from build123d import *

# Parameters (mm, degrees)
EXTRUDE_1_DEPTH     = 45
CUT_EXTRUDE_1_DEPTH = 63.24949799
FILLET_1_R          = 2
FILLET_2_R          = 7
CHAMFER_1_SIZE      = 1


with BuildPart() as part:
    # 草图1 → 拉伸-薄壁1 (new body)
    with BuildSketch(Plane.XY):
        Polygon((0, 0), (0, 30), (35, 30), (35, 25), (5, 25), (5, 0), align=None)
    extrude(amount=EXTRUDE_1_DEPTH)

    # 草图2 → 切除-拉伸1 (cut, through all)
    with BuildSketch(Plane.XZ.offset(-25)):
        with BuildLine():
            Line((27, 35), (27, 10))
            ThreePointArc((27, 10), (22.5, 5.5), (18, 10))
            Line((18, 10), (18, 35))
            ThreePointArc((18, 35), (22.5, 39.5), (27, 35))
        make_face()
    extrude(amount=-CUT_EXTRUDE_1_DEPTH, mode=Mode.SUBTRACT)

    # 圆角1
    fillet_1_edges = [part.edges().sort_by_distance(p)[0] for p in [
        (5, 25, 22.5),
    ]]
    fillet(fillet_1_edges, radius=FILLET_1_R)

    # 圆角2
    fillet_2_edges = [part.edges().sort_by_distance(p)[0] for p in [
        (0, 30, 22.5),
    ]]
    fillet(fillet_2_edges, radius=FILLET_2_R)

    # 倒角1
    chamfer_1_edges = [part.edges().sort_by_distance(p)[0] for p in [
        (2.5, 0, 45),
        (2.5, 0, 0),
        (35, 27.5, 0),
        (35, 27.5, 45),
    ]]
    chamfer(chamfer_1_edges, length=CHAMFER_1_SIZE)


solid = part.part
Design review of the part built by this model. Coordinates are the model's own, in mm. A direction names the side the tool comes from. Give positions to 0.01 mm unless a question says otherwise; leave off trailing zeros. Loops run counter-clockwise (first coordinate to the right, second up) from the corner with the lowest first, then second, coordinate; pieces in that order, holes last. Notation, with made-up numbers: M 50.25,33.5 L 56.25,33.5 A33 ccw 56.25,63.5 Z; hole C -35,12 d7. An arc over 180 degrees is marked long. Answer as a JSON object with one key per item and string values.
Item 1: We need section A-A (x = 22.5). State the section outline as (y, z) points, and give its area (3 significant figures).
Output values:
{"outline": "M 25,0 L 30,0 L 30,5.5 L 25,5.5 Z; M 25,39.5 L 30,39.5 L 30,45 L 25,45 Z", "area": "55.0 mm2"}
Item 2: Machinability: for faces 5 (the face through (18, 27, 22)), 6 (the face through (3, 0, 22)), 7 (the face through (15, 25, 22)), which of the approach directions +Z, -Z, +X, -X, +Y, -Y give a long, thin tool a straight path to every point of the face, cutting with its end or side? Answer none if there is none.
Output values:
{"face 5": "+Y, -Y", "face 6": "+Z, -Z, +X, -X, -Y", "face 7": "+Z, -Z, +X, -Y"}
Item 3: We need section C-C (y = 4.5). State the section outline as (x, z) points.
Output values:
{"outline": "M 0,0 L 5,0 L 5,45 L 0,45 Z"}
Item 4: Mouldability with a two-part tool opening along Z and no side actions: class faces 1 (the face through (12, 26, 0)), 2 (the face through (22.4, 27.5, 39.5)), 3 (the face through (2.1, 28, 22.8)), 4 (the face through (12, 26, 45)) as pulls with the +Z half, pulls with the -Z half, needs draft (parallel to the pull), parting line crosses it, or undercut.
Output values:
{"face 1": "pulls with the -Z half", "face 2": "undercut", "face 3": "needs draft", "face 4": "pulls with the +Z half"}
Item 5: For P1, Ø10, axis at x = 20, z = 25.5, coming from the -Y side; P2, Ø4, axis at y = 28.5, z = 18, coming from the -X side; P3, Ø2, axis at y = 3.5, z = 23, coming from the +X side, all flat-tipped, find the tip position at first contact; note any pin that passes through.
Output values:
{"P1": "stops at y = 25", "P2": "stops at x = 0.94", "P3": "stops at x = 5"}
Item 6: We need section B-B (z = 21.5). State the section outline as (x, y) points, and give its area (3 significant figures).
Output values:
{"outline": "M 0,0 L 5,0 L 5,23 A2 cw 7,25 L 18,25 L 18,30 L 7,30 A7 ccw 0,23 Z; M 27,25 L 35,25 L 35,30 L 27,30 Z", "area": "245 mm2"}
Item 7: Wall thickness on line 1 along X through (y, z) = (26.5, 15); line 2 along X through (y, z) = (18.25, 24); line 3 along Y through (x, z) = (34, 28): over which ranges is each line inside the solid? List them lowest first.
Output values:
{"line 1": "x = 0.94 to 18, 27 to 35", "line 2": "x = 0 to 5", "line 3": "y = 25 to 30"}
